from build123d import *

# Parameters (mm, degrees)
SHANK_PROFILE_0_19_R        = 2.413
SHANK_DEPTH                 = 25.4
SCREWDRIVER_SLOT_DEPTH      = 31.828759505
SCREWDRIVER_SLOT_DEPTH_BACK = 31.828759505
SCREWDRIVER_SLOT_PROFILE_W  = 2.54
SCREWDRIVER_SLOT_PROFILE_H  = 1.27


with BuildPart() as part:
    # Shank Profile Ø0.19 → Shank (new body)
    with BuildSketch(Plane.XY):
        Circle(SHANK_PROFILE_0_19_R)
    extrude(amount=SHANK_DEPTH)

    # Round Head Profile → Round Head (revolve)
    with BuildSketch(Plane(origin=(0, 0, 0), x_dir=(0, 0, -1), z_dir=(1, 0, 0))):
        with BuildLine():
            Line((-25.4, 0), (-25.4, 4.702815049))
            ThreePointArc((-25.4, 4.702815049), (-28.725392412, 3.325392412), (-30.102815049, 0))
            Line((-30.102815049, 0), (-25.4, 0))
        make_face()
    revolve(axis=Axis((0, 0, 25.4), (0, 0, 1)))

    # Screwdriver Slot Profile → Screwdriver Slot (cut, two sides: drawn at the far end of the back side and taken through both)
    with BuildSketch(Plane(origin=(0, 0, 0), x_dir=(0, 0, -1), z_dir=(1, 0, 0)).offset(-SCREWDRIVER_SLOT_DEPTH_BACK)):
        with Locations((-29.795276549, 0)):
            Rectangle(SCREWDRIVER_SLOT_PROFILE_W, SCREWDRIVER_SLOT_PROFILE_H)
    extrude(amount=SCREWDRIVER_SLOT_DEPTH + SCREWDRIVER_SLOT_DEPTH_BACK, mode=Mode.SUBTRACT)


solid = part.part
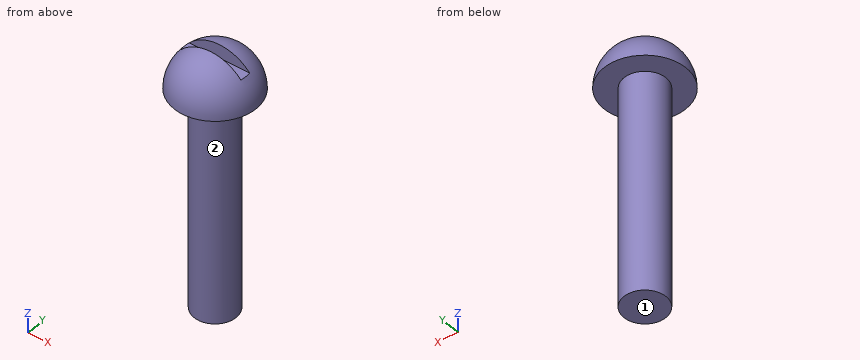
Could you check a few things on this model? Use its own coordinates, in mm. Face numbers are marked on the shaded views. A direction names the side the tool comes from. Give positions to 0.01 mm unless a question says otherwise; leave off trailing zeros. Write each loop counter-clockwise with the first axis right and the second up, starting at its lowest first coordinate (ties: lowest second). Pieces come first, ordered by that corner, then holes. Notation, with made-up numbers: (86.25, 3.5) - (94.25, 3.5) arc R11 cw to (94.25, 21.5) - close; hole circle Ø11 at (21.5, 76.25). An arc over 180 degrees is marked (long way). Use CSV: the item, a comma, the result in double quotes. Start each with the question number.
Item 1: If I drill on line 1 along Z through (x, y) = (-3.25, -0.5); line 2 along Z through (x, y) = (-0.75, 0.25); line 3 along X through (y, z) = (-1.5, 16.5), over which ranges is the centre line in solid material (lowest first)?
Item 2: I want a section at C-C, the plane z = 3. Please give me the cut outline in (x, y).
Item 3: I want a section at A-A, the plane y = 0. Please give me the cut outline in (x, z), then the cut area to 3 significant figures.
Item 4: I want a section at D-D, the plane x = 1.5. Please give me the cut outline in (y, z) (3 decimals), then the cut area to 3 significant figures.
Item 5: I want a section at B-B, the plane x = 0. Please give me the cut outline in (y, z) (3 decimals).
Item 6: I'm going to push flat-ended pins straight in: pin 1 (1.7 mm diameter, centred on x = 0, z = 29, fed in from -Y); pin 2 (2 mm diameter, centred on y = -1, z = 17.5, fed in from -X); pin 3 (1 mm diameter, centred on x = -2.5, y = 0.5, fed in from +Z). Where does each tip first touch, or does it pass through?
Item 7: For the marked faces 1 and 2, which set-ups out of +Z, -Z, +X, -X, +Y, -Y let a thin tool reach every point of the face, with its end or its side?
Findings:
1,line 1,"z = 25.4 to 28.53"
1,line 2,"z = 0 to 28.53"
1,line 3,"x = -1.89 to 1.89"
2,outline,"circle Ø4.83 at (0, 0)"
3,outline,"(-4.7, 25.4) - (-2.41, 25.4) - (-2.41, 0) - (2.41, 0) - (2.41, 25.4) - (4.7, 25.4) arc R4.7 ccw to (3.51, 28.53) - (-3.51, 28.53) arc R4.7 ccw to start"
3,area,"150 mm2"
4,outline,"(-4.457, 25.4) - (-1.89, 25.4) - (-1.89, 0) - (1.89, 0) - (1.89, 25.4) - (4.457, 25.4) arc R4.457 ccw to (0.635, 29.812) - (0.635, 28.525) - (-0.635, 28.525) - (-0.635, 29.812) arc R4.457 ccw to start"
4,area,"126 mm2"
5,outline,"(-4.703, 25.4) - (-2.413, 25.4) - (-2.413, 0) - (2.413, 0) - (2.413, 25.4) - (4.703, 25.4) arc R4.703 ccw to (0.635, 30.06) - (0.635, 28.525) - (-0.635, 28.525) - (-0.635, 30.06) arc R4.703 ccw to start"
6,pin 1,"stops at y = -3.81"
6,pin 2,"stops at x = -2.41"
6,pin 3,"stops at z = 29.6"
7,face 1,"-Z, +X, -X, +Y, -Y"
7,face 2,"-Z"
